For this review, take the finished solid that the model builds, in its own axes (mm). Face numbers are marked on the shaded views. A direction names the side the tool comes from. Give positions to 0.01 mm unless a question says otherwise; leave off trailing zeros. Loops run counter-clockwise (first coordinate to the right, second up) from the corner with the lowest first, then second, coordinate; pieces in that order, holes last. Notation, with made-up numbers: (59, 49) -> (111, 49) arc R16 ccw to (111, 57) -> close; hole circle Ø4 at (-9.75, -24). An arc over 180 degrees is marked (long way). One line per question, with ' | ' between items. Start each with the question number.
(1) Consider section B-B (x = 3). Write out the cut boundary in (y, z).
(2) Tool access review of the marked faces 1, 2, 3, 4 and 5: name each direction out of +Z, -Z, +X, -X, +Y, -Y from which nothing blocks a thin tool from reaching the whole face with its end or side.
(3) Wall thickness on probe 1 along Y at (x, z) = (11.25, 0); probe 2 along X at (y, z) = (-15, -30.5); probe 3 along X at (y, z) = (19, 9): over which ranges is each line inside the solid? List them lowest first.
(4) Draft analysis for pull direction X (two halves, no side actions). For the marked faces 6, 7 and 8, state which applies: +X half, -X half, draft (parallel to the pull), parting line (faces both ways), or undercut.
(5) Consider section A-A (x = -4.5). Write out the cut boundary in (y, z).
(6) Insertion check: P1, Ø1, axis at x = 1, y = -18, coming from the +Z side; P2, Ø12, axis at x = -4, z = 22, coming from the -Y side; P3, Ø4, axis at x = -2.5, y = -18, coming from the +Z side. Each pin has a flat end and moves straight along its axis. Give the tip position at first contact, or say it passes through.
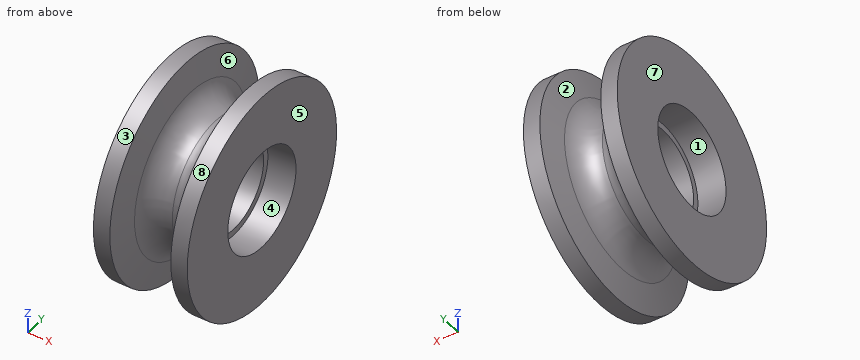
from build123d import *


with BuildPart() as part:
    # Sketch1 → Revolve1 (revolve)
    with BuildSketch(Plane.XY, mode=Mode.PRIVATE) as revolve1_sk:
        with BuildLine():
            Line((-6, 14), (6, 14))
            Line((6, 14), (6, 16))
            Line((6, 16), (15, 16))
            Line((15, 16), (15, 35))
            Line((15, 35), (9.746098753, 35))
            Line((9.746098753, 35), (7.810368057, 26.268483088))
            ThreePointArc((7.810368057, 26.268483088), (5.007387777, 21.760924135), (0, 20))
            ThreePointArc((0, 20), (-5.007387777, 21.760924135), (-7.810368057, 26.268483088))
            Line((-7.810368057, 26.268483088), (-9.746098753, 35))
            Line((-9.746098753, 35), (-15, 35))
            Line((-15, 35), (-15, 16))
            Line((-15, 16), (-6, 16))
            Line((-6, 16), (-6, 14))
        make_face()
    revolve(revolve1_sk.sketch.rotate(Axis((0, 0, 0), (1, 0, 0)), 90), axis=Axis((0, 0, 0), (1, 0, 0)))


solid = part.part
A:
1) outline: circle Ø41.17 at (0, 0); hole circle Ø28 at (0, 0)
2) face 1: -X | face 2: none | face 3: +X, -X | face 4: +X | face 5: +Z, -Z, +X, +Y, -Y
3) probe 1: y = -35 to -16, 16 to 35 | probe 2: x = -15 to -9.52, 9.52 to 15 | probe 3: x = -15 to -3.92, 3.92 to 15
4) face 6: undercut | face 7: -X half | face 8: draft
5) outline: circle Ø42.77 at (0, 0); hole circle Ø28 at (0, 0)
6) P1: stops at z = 9.82 | P2: stops at y = -28.53 | P3: stops at z = 12.97
